```python
from build123d import *

# Parameters (mm, degrees)
SKETCH1_R               = 6
BOSS_EXTRUDE1_DEPTH     = 130
CUT_EXTRUDE1_DEPTH      = 131.276628756
CUT_EXTRUDE1_DEPTH_BACK = 131.276628756
SKETCH3_R               = 2.75
CHAMFER1_SIZE           = 1
SKETCH5_W               = 10
SKETCH5_H               = 20
CUT_EXTRUDE2_DEPTH      = 1.5
MIRROR2_COPY_1_SKETCH_W = 10
MIRROR2_COPY_1_SKETCH_H = 20
MIRROR2_COPY_1_DEPTH    = 1.5
SKETCH7_R               = 6
SKETCH7_R_2             = 5.75
CUT_EXTRUDE3_DEPTH      = 1


with BuildPart() as part:
    # Sketch1 → Boss-Extrude1 (new body)
    with BuildSketch(Plane(origin=(0, 0, 0), x_dir=(1, 0, 0), z_dir=(0, 1, 0))):
        with Locations(Location((0, 0, 0), (0, 0, 270))):
            Circle(SKETCH1_R)
    extrude(amount=BOSS_EXTRUDE1_DEPTH)

    # Sketch3 → Cut-Extrude1 (cut, two sides: drawn at the far end of the back side and taken through both)
    with BuildSketch(Plane(origin=(0, 0, 0), x_dir=(0, 0, -1), z_dir=(1, 0, 0)).offset(-CUT_EXTRUDE1_DEPTH_BACK)):
        with Locations((0, 125)):
            Circle(SKETCH3_R)
        with Locations((0, 5)):
            Circle(SKETCH3_R)
    extrude(amount=CUT_EXTRUDE1_DEPTH + CUT_EXTRUDE1_DEPTH_BACK, mode=Mode.SUBTRACT)

    # Chamfer1
    chamfer1_edges = [part.edges().sort_by_distance(p)[0] for p in [
        (0, 0, -6),
        (0, 130, -6),
    ]]
    chamfer(chamfer1_edges, length=CHAMFER1_SIZE)

    # Sketch5 → Cut-Extrude2 (cut)
    with BuildSketch(Plane(origin=(6, 0, 0), x_dir=(0, 0, -1), z_dir=(1, 0, 0))):
        Rectangle(SKETCH5_W, SKETCH5_H)
    cut_extrude2 = extrude(amount=-CUT_EXTRUDE2_DEPTH, mode=Mode.SUBTRACT)

    # Mirror1: Cut-Extrude2 across plane
    add(cut_extrude2.mirror(Plane(origin=(0, 0, 0), x_dir=(0, 0, 1), z_dir=(1, 0, 0))), mode=Mode.SUBTRACT)

    # Mirror2: Cut-Extrude2 across plane
    add(cut_extrude2.mirror(Plane(origin=(0, 65, 0), x_dir=(0, 0, 1), z_dir=(0, -1, 0))), mode=Mode.SUBTRACT)

    # Mirror2 copy 1 sketch → Mirror2 copy 1 (cut)
    with BuildSketch(Plane(origin=(-6, 130, 0), x_dir=(0, 0, -1), z_dir=(-1, 0, 0))):
        Rectangle(MIRROR2_COPY_1_SKETCH_W, MIRROR2_COPY_1_SKETCH_H)
    extrude(amount=-MIRROR2_COPY_1_DEPTH, mode=Mode.SUBTRACT)

    # Sketch7 → Cut-Extrude3 (cut)
    with BuildSketch(Plane(origin=(0, 104, 0), x_dir=(1, 0, 0), z_dir=(0, 1, 0))):
        with Locations(Location((0, 0, 0), (0, 0, 138.590377891))):
            Circle(SKETCH7_R)
        with Locations(Location((0, 0, 0), (0, 0, 270))):
            Circle(SKETCH7_R_2, mode=Mode.SUBTRACT)
    cut_extrude3 = extrude(amount=CUT_EXTRUDE3_DEPTH, mode=Mode.SUBTRACT)

    # Mirror3: Cut-Extrude3 across plane
    add(cut_extrude3.mirror(Plane(origin=(0, 65, 0), x_dir=(0, 0, 1), z_dir=(0, -1, 0))), mode=Mode.SUBTRACT)


solid = part.part
```
Source: CAD feature listing. Evaluate the final solid. Frame: model axes, mm. A direction names the side the tool comes from. Coordinates: 2 decimals unless noted, no trailing zeros. Loops run counter-clockwise (first coordinate to the right, second up) from the corner with the lowest first, then second, coordinate; pieces in that order, holes last. Notation, with made-up numbers: (42.25, 35.25) - (59.25, 35.25) arc R30 ccw to (59.25, 61.25) - close; hole circle Ø9 at (44.5, 69.25). An arc over 180 degrees is marked (long way). Answer as CSV lines item,"result".
1. Reachability of faces 4 (the flat face through (4.5, 122.7, 1.8)), 5 (the cylindrical face through (4.85, 25.51, 3.09)), 6 (the flat face through (-4.5, 7.3, 1.8)), 7 (the flat face through (4.5, 7.3, 1.8)) from +Z, -Z, +X, -X, +Y, -Y: full face, straight path, thin tool, end or side. Return the list, or none.
Established:
face 4,"+Z, -Z, +X, +Y"
face 5,"none"
face 6,"+Z, -Z, -X, -Y"
face 7,"+Z, -Z, +X, -Y"
2. Section C-C (z = 0). Count the separate pieces of the cut face and the enclosed holes in it, then the cut area to 3 significant figures.
Established:
separate pieces,"3"
enclosed holes,"0"
area,"1,400 mm2"
3. Section B-B (y = 5). Return loops of the section in (x, z).
Established:
outline,"(-4.5, -3.97) arc R6 ccw to (4.5, -3.97) - (4.5, -2.75) - (-4.5, -2.75) - close; (-4.5, 2.75) - (4.5, 2.75) - (4.5, 3.97) arc R6 ccw to (-4.5, 3.97) - close"
4. Mould query, pull axis Z, two halves, no side actions, for faces 1 (the cylindrical face through (-0.063, 2.315, 0.596)), 2 (the cylindrical face through (0, 15, -6)), 3 (the conical face through (0.1, 0.2, -5.2)). Classes: released by +Z, released by -Z, zero draft, split by the parting line, or undercut.
Established:
face 1,"undercut"
face 2,"split by the parting line"
face 3,"released by -Z"
5. Contact query for flat-ended pins moving along their axis: pin 1 (5 mm diameter, centred on x = 2, y = 52.5, fed in from -Z); pin 2 (4 mm diameter, centred on x = 3, y = 56.5, fed in from +Z); pin 3 (1.2 mm diameter, centred on x = 5.5, z = -1.5, fed in from -Y); pin 4 (7 mm diameter, centred on y = 5, z = 0, fed in from -X). Output: stop coordinate, or through.
Established:
pin 1,"stops at z = -6"
pin 2,"stops at z = 5.92"
pin 3,"stops at y = 10"
pin 4,"stops at x = -4.5"
6. Section A-A (x = 0). Return loops of the section in (y, z), then the cut area to 3 significant figures.
Established:
outline,"(0, -5) - (1, -6) - (25, -6) - (25, -5.75) - (26, -5.75) - (26, -6) - (104, -6) - (104, -5.75) - (105, -5.75) - (105, -6) - (129, -6) - (130, -5) - (130, 5) - (129, 6) - (105, 6) - (105, 5.75) - (104, 5.75) - (104, 6) - (26, 6) - (26, 5.75) - (25, 5.75) - (25, 6) - (1, 6) - (0, 5) - close; hole circle Ø5.5 at (5, 0); hole circle Ø5.5 at (125, 0)"
area,"1,510 mm2"
7. Section D-D (y = 45.5). Return loops of the section in (x, z), then the cut area to 3 significant figures.
Established:
outline,"circle Ø12 at (0, 0)"
area,"113 mm2"
8. Ray query, line 1 (Y direction, x = -1, z = 0); line 2 (Y direction, x = 5, z = -3.25); line 3 (X direction, y = 48.5, z = -4.5). Return the intervals inside material, ascending.
Established:
line 1,"y = 0 to 2.25, 7.75 to 122.25, 127.75 to 130"
line 2,"y = 10 to 25, 26 to 104, 105 to 120"
line 3,"x = -3.97 to 3.97"
